from build123d import *

# Parameters (mm, degrees)
MUG_WALL_DEPTH            = 22.5
MUG_BOTTOM_DEPTH          = 1.5
BOTTOM_EDGE_FILLET_R0_9_R = 0.9
HANDLE_DEPTH              = 1.5
HANDLE_EDGE_FILLET_R1_2_R = 1.2


with BuildPart() as part:
    # Wall Profile Octagon → Mug Wall (new, symmetric)
    with BuildSketch(Plane(origin=(0, 0, 0), x_dir=(1, 0, 0), z_dir=(0, 1, 0))):
        Polygon((21.848632739, -9.05), (21.848632739, 9.05), (9.05, 21.848632739), (-9.05, 21.848632739), (-21.848632739, 9.05), (-21.848632739, -9.05), (-9.05, -21.848632739), (9.05, -21.848632739), align=None)
        Polygon((19.8, 8.201428535), (8.201428535, 19.8), (-8.201428535, 19.8), (-19.8, 8.201428535), (-19.8, -8.201428535), (-8.201428535, -19.8), (8.201428535, -19.8), (19.8, -8.201428535), align=None, mode=Mode.SUBTRACT)
    extrude(amount=MUG_WALL_DEPTH, both=True)

    # Bottom Profile Octagon → Mug Bottom (add)
    with BuildSketch(Plane(origin=(0, -20.5, 0), x_dir=(1, 0, 0), z_dir=(0, 1, 0))):
        Polygon((-19.8, 8.201428535), (-19.8, -8.201428535), (-8.201428535, -19.8), (8.201428535, -19.8), (19.8, -8.201428535), (19.8, 8.201428535), (8.201428535, 19.8), (-8.201428535, 19.8), align=None)
    extrude(amount=MUG_BOTTOM_DEPTH)

    # Bottom Edge Fillet R0.9
    bottom_edge_fillet_r0_9_edges = [part.edges().sort_by_distance(p)[0] for p in [
        (-14.000714267, -20.5, -14.000714267),
        (-19.8, -20.5, 0),
        (-14.000714267, -20.5, 14.000714267),
        (0, -20.5, 19.8),
        (14.000714267, -20.5, 14.000714267),
        (19.8, -20.5, 0),
        (14.000714267, -20.5, -14.000714267),
        (0, -20.5, -19.8),
    ]]
    fillet(bottom_edge_fillet_r0_9_edges, radius=BOTTOM_EDGE_FILLET_R0_9_R)

    # Handle Profile → Handle (add, symmetric)
    with BuildSketch(Plane.XY):
        with BuildLine():
            Line((21.848632739, -12.051874881), (34.972961948, -4.18790751))
            ThreePointArc((34.972961948, -4.18790751), (38.548632739, 10.078647028), (24.282078201, 13.65431782))
            Line((24.282078201, 13.65431782), (21.848632739, 12.196221531))
            Line((21.848632739, 12.196221531), (21.848632739, 14.644346649))
            Line((21.848632739, 14.644346649), (23.202710131, 15.455696338))
            ThreePointArc((23.202710131, 15.455696338), (40.350011258, 11.158015099), (36.052330019, -5.989286029))
            Line((36.052330019, -5.989286029), (21.848632739, -14.5))
            Line((21.848632739, -14.5), (21.848632739, -12.051874881))
        make_face()
    extrude(amount=HANDLE_DEPTH, both=True)

    # Handle Edge Fillet R1.2
    handle_edge_fillet_r1_2_edges = [part.edges().sort_by_distance(p)[0] for p in [
        (28.950481379, -10.244643014, -1.5),
        (40.350011258, 11.158015099, -1.5),
        (22.525671435, 15.050021494, -1.5),
        (28.950481379, -10.244643014, 1.5),
        (40.350011258, 11.158015099, 1.5),
        (22.525671435, 15.050021494, 1.5),
    ]]
    fillet(handle_edge_fillet_r1_2_edges, radius=HANDLE_EDGE_FILLET_R1_2_R)


solid = part.part
Verification items for the finished model (mm, model axes). A direction names the side the tool comes from. Coordinates: 2 decimals unless noted, no trailing zeros. Order: outer loops, then holes, each group sorted by start corner. A loop starts at its lowest first (then second) coordinate and runs counter-clockwise, first axis right, second up. Notation, with made-up numbers: M -16.75,66.5 L 12.25,66.5 A21 ccw 12.25,102.5 Z; hole C 53.5,61 d9. An arc over 180 degrees is marked long. Return JSON: item names as keys, results as strings.
1) Cross-section at C-C, the plane y = 8.5. Count the separate pieces of the cut face and the enclosed holes in it, and give its area (3 significant figures).
Answer list:
{"separate pieces": "2", "enclosed holes": "1", "area": "289 mm2"}
2) Release check for a two-part mould opening along X. For faces 1 (the cylindrical face through (28.67, -9.99, 1.16)), 2 (the flat face through (-14, 2, 14)), 3 (the flat face through (-14, -22, -14)), 4 (the flat face through (14.5, -22.5, 14.5)) record: +X half, -X half, draft (parallel to the pull), parting line (faces both ways), or undercut.
Answer list:
{"face 1": "+X half", "face 2": "undercut", "face 3": "undercut", "face 4": "draft"}
3) Cross-section at B-B, the plane z = -5. Record the boundary of the cut face in (x, y).
Answer list:
{"outline": "M -21.85,-22.5 L -19.8,-22.5 L -19.8,-21.4 A0.9 cw -18.9,-20.5 L 18.9,-20.5 A0.9 cw 19.8,-21.4 L 19.8,-22.5 L 21.85,-22.5 L 21.85,22.5 L 19.8,22.5 L 19.8,-19 L -19.8,-19 L -19.8,22.5 L -21.85,22.5 Z"}
4) Gauge pin test, flat ends, axial feed: pin 1 (0.6 mm diameter, centred on y = -22, z = -1.5, fed in from +X); pin 2 (6 mm diameter, centred on x = 21, y = 2.5, fed in from +Z); pin 3 (19 mm diameter, centred on x = -7, z = 7, fed in from -Y). Record the tip position at first contact, or that the pin passes through.
Answer list:
{"pin 1": "x = 21.85", "pin 2": "z = 12.9", "pin 3": "y = -20.65"}
5) Cross-section at A-A, the plane x = 2.5. Record the boundary of the cut face in (y, z), and give its area (3 significant figures).
Answer list:
{"outline": "M -22.5,-21.85 L 22.5,-21.85 L 22.5,-19.8 L -19,-19.8 L -19,19.8 L 22.5,19.8 L 22.5,21.85 L -22.5,21.85 L -22.5,19.8 L -21.4,19.8 A0.9 cw -20.5,18.9 L -20.5,-18.9 A0.9 cw -21.4,-19.8 L -22.5,-19.8 Z", "area": "244 mm2"}
6) Thickness scan on L1, parallel to Z at x = 3, y = -2; L2, parallel to X at y = -1, z = 0.5. Record the ranges inside material, lowest first. Write a range as [from, to].
Answer list:
{"L1": "[-21.85, -19.8], [19.8, 21.85]", "L2": "[-21.85, -19.8], [19.8, 21.85], [38.3, 40.72]"}
7) Access from +Z, -Z, +X, -X, +Y, -Y to the whole of each face (thin tool, end or side, straight path). Record for faces 5 (the flat face through (40, 7, 1.5)), 6 (the cylindrical face through (13.74, -20.77, -13.9)), 7 (the flat face through (23.082, 12.935, 0.021)), 8 (the flat face through (14, 2, 14)).
Answer list:
{"face 5": "+Z, +X, +Y, -Y", "face 6": "-Y", "face 7": "+Z, -Z", "face 8": "+Y"}
